Here's how the part is built. I have some questions about the finished solid (model axes, mm). Face numbers are marked on the shaded views. A direction names the side the tool comes from. Coordinates: 2 decimals unless noted, no trailing zeros. Write each loop counter-clockwise with the first axis right and the second up, starting at its lowest first coordinate (ties: lowest second). Pieces come first, ordered by that corner, then holes. Notation, with made-up numbers: M 28.5,-14 L 50.5,-14 A24 cw 50.5,2 Z; hole C 23.5,81 d4. An arc over 180 degrees is marked long. Use a Markdown table: item, result.
```python
from build123d import *

# Parameters (mm, degrees)
CHAMFER1_SIZE       = 1
CHAMFER2_SIZE       = 1
BOSS_EXTRUDE1_DEPTH = 9


with BuildPart() as part:
    # Sketch1 → Revolve1 (revolve)
    with BuildSketch(Plane.XY, mode=Mode.PRIVATE) as revolve1_sk:
        Polygon((-21.47270101, 0), (-21.47270101, 9), (1.52729899, 9), (1.52729899, 7), (23.52729899, 7), (23.52729899, 0), align=None)
    revolve(revolve1_sk.sketch.rotate(Axis((-65.318854856, 0, 0), (1, 0, 0)), 90), axis=Axis((-65.318854856, 0, 0), (1, 0, 0)))

    # Chamfer1
    chamfer1_edges = [part.edges().sort_by_distance(p)[0] for p in [
        (23.52729899, 0, -7),
    ]]
    chamfer(chamfer1_edges, length=CHAMFER1_SIZE)

    # Chamfer2
    chamfer2_edges = [part.edges().sort_by_distance(p)[0] for p in [
        (-21.47270101, 0, -9),
    ]]
    chamfer(chamfer2_edges, length=CHAMFER2_SIZE)

    # Sketch3 → Boss-Extrude1 (add)
    with BuildSketch(Plane.ZY.offset(21.47270101)):
        with BuildLine():
            Line((4, 0), (2.543967169, 5.433988502))
            ThreePointArc((2.543967169, 5.433988502), (0, 6), (-2.543967169, 5.433988502))
            Line((-2.543967169, 5.433988502), (-4, 0))
            Line((-4, 0), (-2.543967169, -5.433988502))
            ThreePointArc((-2.543967169, -5.433988502), (0, -6), (2.543967169, -5.433988502))
            Line((2.543967169, -5.433988502), (4, 0))
        make_face()
    extrude(amount=BOSS_EXTRUDE1_DEPTH)


solid = part.part
```
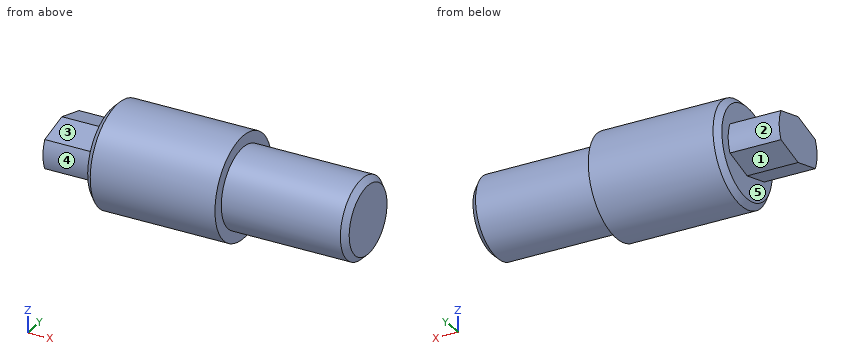
1. Will these pins go through, and if not, where does the flat tip stop? pin 1 Ø4 at (x, z) = (-21, 6) entering from +Y; pin 2 Ø4 at (y, z) = (-2.5, 4) entering from -X; pin 3 Ø1.5 at (x, y) = (-11, -5) entering from +Z; pin 4 Ø3 at (x, z) = (4.5, 0.5) entering from +Y.
Answers follow:
| item | result |
|---|---|
| pin 1 | stops at y = 8.03 |
| pin 2 | stops at x = -30.47 |
| pin 3 | stops at z = 7.93 |
| pin 4 | stops at y = 7 |
2. I need wall thicknesses on probe 1 along Y at (x, z) = (17.5, 0); probe 2 along X at (y, z) = (-0.5, 5); probe 3 along X at (y, z) = (4.5, -5.5). Which ranges of each line are inside material? Lowest first, please.
Answers follow:
| item | result |
|---|---|
| probe 1 | y = -7 to 7 |
| probe 2 | x = -21.47 to 23.53 |
| probe 3 | x = -21.47 to 1.53 |
3. Which directions (+Z, -Z, +X, -X, +Y, -Y) give clear straight access to the entire face, cutting with the end or side of a thin tool? Please do the marked faces 1, 2, 3, 4 and 5.
Answers follow:
| item | result |
|---|---|
| face 1 | -Z, -X, +Y |
| face 2 | -X, +Y |
| face 3 | +Z, -X, -Y |
| face 4 | -X, -Y |
| face 5 | -X |
4. Suppose I cut it at D-D on x = -3. Write out the boundary of the cut face in (y, z).
Answers follow:
| item | result |
|---|---|
| outline | C 0,0 d18 |
5. Suppose I cut it at B-B on z = 0. Write out the boundary of the cut face in (x, y).
Answers follow:
| item | result |
|---|---|
| outline | M -30.47,-6 L -21.47,-6 L -21.47,-8 L -20.47,-9 L 1.53,-9 L 1.53,-7 L 22.53,-7 L 23.53,-6 L 23.53,6 L 22.53,7 L 1.53,7 L 1.53,9 L -20.47,9 L -21.47,8 L -21.47,6 L -30.47,6 Z |
6. Suppose I cut it at A-A on x = -26. Write out the boundary of the cut face in (y, z), and give its area (3 significant figures).
Answers follow:
| item | result |
|---|---|
| outline | M -5.43,-2.54 L 0,-4 L 5.43,-2.54 A6 ccw 5.43,2.54 L 0,4 L -5.43,2.54 A6 ccw Z |
| area | 75.0 mm2 |
7. Suppose I cut it at C-C on x = 12.5. Write out the boundary of the cut face in (y, z), and give its area (3 significant figures).
Answers follow:
| item | result |
|---|---|
| outline | C 0,0 d14 |
| area | 154 mm2 |
